```python
from build123d import *

# Parameters (mm, degrees)
SKETCH1_W           = 80
SKETCH1_H           = 80
SKETCH1_R           = 12
SKETCH1_R_2         = 4.5
BOSS_EXTRUDE1_DEPTH = 8
CHAMFER1_SIZE       = 5


with BuildPart() as part:
    # Sketch1 → Boss-Extrude1 (new body)
    with BuildSketch(Plane.XY):
        with Locations((-1.114398958, 9.473684211)):
            Rectangle(SKETCH1_W, SKETCH1_H)
        with Locations((-1.114398958, 9.473684211)):
            Circle(SKETCH1_R, mode=Mode.SUBTRACT)
        with Locations((-30.114398958, 38.473684211)):
            Circle(SKETCH1_R_2, mode=Mode.SUBTRACT)
        with Locations((-30.114398958, -19.526315789)):
            Circle(SKETCH1_R_2, mode=Mode.SUBTRACT)
        with Locations((27.885601042, -19.526315789)):
            Circle(SKETCH1_R_2, mode=Mode.SUBTRACT)
        with Locations((27.885601042, 38.473684211)):
            Circle(SKETCH1_R_2, mode=Mode.SUBTRACT)
    extrude(amount=BOSS_EXTRUDE1_DEPTH)

    # Chamfer1
    chamfer1_edges = [part.edges().sort_by_distance(p)[0] for p in [
        (-41.114398958, 49.473684211, 4),
        (38.885601042, 49.473684211, 4),
        (38.885601042, -30.526315789, 4),
        (-41.114398958, -30.526315789, 4),
    ]]
    chamfer(chamfer1_edges, length=CHAMFER1_SIZE)


solid = part.part
```
The listing builds one solid part. Answer for the finished solid, in the listing's coordinates (mm). Coordinates: 2 decimals unless noted, no trailing zeros. Order: outer loops, then holes, each group sorted by start corner. A loop starts at its lowest first (then second) coordinate and runs counter-clockwise, first axis right, second up. Notation, with made-up numbers: M 33,60.25 L 88,60.25 A25 cw 88,93.25 Z; hole C 72,23 d9. An arc over 180 degrees is marked long. Answer as a JSON object with one key per item and string values. Group by question number.
1. Determine the mould class of faces 1 (the flat face through (-38.58, 47.01, 3.94)), 2 (the flat face through (38.886, 9, 4)), 3 (the cylindrical face through (26.91, -23.92, 3.94)), 4 (the flat face through (-2, -30.526, 4)) for opening direction Y: released by +Y, released by -Y, zero draft, split by the parting line, or undercut.
2. Section C-C on y = 41 is taken. Write down the section's boundary in (x, z), then the cut area to 3 significant figures.
3. Straight lines are drawn through the part: line 1 (Y direction, x = 28.5, z = 4.25); line 2 (Y direction, x = -31.5, z = 1.25); line 3 (X direction, y = -19, z = 7.75). For each, find the intervals that lie inside material, in ascending order.
4. Section D-D on z = 2.5 is taken. Write down the section's boundary in (x, y).
5. Section B-B on x = -31 is taken. Write down the section's boundary in (y, z).
6. Section A-A on y = 0 is taken. Write down the section's boundary in (x, z).
Values follow:
{
 "1": {"face 1": "released by +Y", "face 2": "zero draft", "face 3": "undercut", "face 4": "released by -Y"},
 "2": {"outline": "M -41.11,0 L -33.84,0 L -33.84,8 L -41.11,8 Z; M -26.39,0 L 24.16,0 L 24.16,8 L -26.39,8 Z; M 31.61,0 L 38.89,0 L 38.89,8 L 31.61,8 Z", "area": "521 mm2"},
 "3": {"line 1": "-30.53 to -23.98, -15.07 to 34.02, 42.93 to 49.47", "line 2": "-30.53 to -23.81, -15.24 to 34.19, 42.76 to 49.47", "line 3": "-41.11 to -34.58, -25.65 to 23.42, 32.35 to 38.89"},
 "4": {"outline": "M -41.11,-25.53 L -36.11,-30.53 L 33.89,-30.53 L 38.89,-25.53 L 38.89,44.47 L 33.89,49.47 L -36.11,49.47 L -41.11,44.47 Z; hole C -30.11,-19.53 d9; hole C -30.11,38.47 d9; hole C -1.11,9.47 d24; hole C 27.89,-19.53 d9; hole C 27.89,38.47 d9"},
 "5": {"outline": "M -30.53,0 L -23.94,0 L -23.94,8 L -30.53,8 Z; M -15.11,0 L 34.06,0 L 34.06,8 L -15.11,8 Z; M 42.89,0 L 49.47,0 L 49.47,8 L 42.89,8 Z"},
 "6": {"outline": "M -41.11,0 L -8.48,0 L -8.48,8 L -41.11,8 Z; M 6.25,0 L 38.89,0 L 38.89,8 L 6.25,8 Z"}
}
